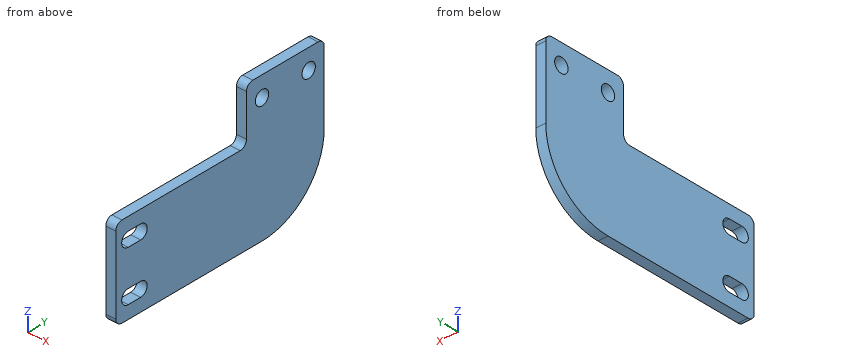
from build123d import *

# Parameters (mm, degrees)
EXTRUDE_1_DEPTH             = 3
EXTRUDE_2_DEPTH             = 3
CUT_EXTRUDE_1_DEPTH         = 3
FILLET_2_R                  = 2
HOLE_WIZARD_4_3_4_3_1_D     = 4.3
HOLE_WIZARD_4_3_4_3_1_DEPTH = 10.1
HOLE_WIZARD_4_3_4_3_1_TIP   = 1.291850331
EXTRUDE_3_DEPTH             = 3
PATTERN_LINEAR_1_COUNT      = 2
PATTERN_LINEAR_1_PITCH      = 24
SKETCH_8_W                  = 24.221203915
SKETCH_8_H                  = 43.975746473
CUT_EXTRUDE_2_DEPTH         = 10
SKETCH_9_W                  = 8.594531195
SKETCH_9_H                  = 29.155429328
CUT_EXTRUDE_3_DEPTH         = 10
FILLET_3_R                  = 2
FILLET_4_R                  = 20


with BuildPart() as part:
    # 草图1 → 凸台-拉伸1 (new body)
    with BuildSketch(Plane(origin=(0, 0, 0), x_dir=(0, 0, -1), z_dir=(1, 0, 0))):
        Polygon((-12.5, 6), (-6, 6), (-6, 61), (6, 61), (6, 6), (12.5, 6), (12.5, -6), (-12.5, -6), align=None)
    extrude(amount=EXTRUDE_1_DEPTH)

    # 草图2 → 凸台-拉伸2 (add)
    with BuildSketch(Plane.ZY):
        Polygon((-6, 61), (-12.5, 6), (12.5, 6), (6, 61), align=None)
    extrude(amount=-EXTRUDE_2_DEPTH)

    # 草图3 → 切除-拉伸1 (cut)
    with BuildSketch(Plane.ZY):
        with BuildLine():
            Line((-5.4, 2), (-5.4, -2))
            ThreePointArc((-5.4, -2), (-7.5, -4.1), (-9.6, -2))
            Line((-9.6, -2), (-9.6, 2))
            ThreePointArc((-9.6, 2), (-7.5, 4.1), (-5.4, 2))
        make_face()
        with BuildLine():
            Line((5.4, 2), (5.4, -2))
            ThreePointArc((5.4, -2), (7.5, -4.1), (9.6, -2))
            Line((9.6, -2), (9.6, 2))
            ThreePointArc((9.6, 2), (7.5, 4.1), (5.4, 2))
        make_face()
    cut_extrude_1 = extrude(amount=-CUT_EXTRUDE_1_DEPTH, mode=Mode.SUBTRACT)

    # 圆角2
    fillet_2_edges = [part.edges().sort_by_distance(p)[0] for p in [
        (1.5, -6, -12.5),
        (1.5, -6, 12.5),
    ]]
    fillet(fillet_2_edges, radius=FILLET_2_R)

    # Ø4.3 (4.3) 直径孔1
    with Locations(Plane.ZY):
        with Locations((0, 56), (0, 41)):
            Hole(HOLE_WIZARD_4_3_4_3_1_D / 2, depth=HOLE_WIZARD_4_3_4_3_1_DEPTH)
            with Locations((0, 0, -(HOLE_WIZARD_4_3_4_3_1_DEPTH + HOLE_WIZARD_4_3_4_3_1_TIP / 2))):  # 118° drill point
                Cone(0, HOLE_WIZARD_4_3_4_3_1_D / 2, HOLE_WIZARD_4_3_4_3_1_TIP, mode=Mode.SUBTRACT)

    # 草图7 → 凸台-拉伸3 (add)
    with BuildSketch(Plane.ZY):
        Polygon((-3.566854944, 61), (-37.5, 61), (-37.5, -6), (-10.5, -6), (-10.5, 36), (-3.566854944, 36), align=None)
    extrude(amount=-EXTRUDE_3_DEPTH)

    # 阵列(线性)1: 切除-拉伸1 ×2
    with Locations(*[(0, 0, -i * PATTERN_LINEAR_1_PITCH) for i in range(1, PATTERN_LINEAR_1_COUNT)]):
        add(cut_extrude_1, mode=Mode.SUBTRACT)

    # 草图8 → 切除-拉伸2 (cut)
    with BuildSketch(Plane.ZY):
        with Locations((1.610601958, 14.012126763)):
            Rectangle(SKETCH_8_W, SKETCH_8_H)
    extrude(amount=-CUT_EXTRUDE_2_DEPTH, mode=Mode.SUBTRACT)

    # 草图9 → 切除-拉伸3 (cut)
    with BuildSketch(Plane.ZY):
        with Locations((10.297265598, 46.422285336)):
            Rectangle(SKETCH_9_W, SKETCH_9_H)
    extrude(amount=-CUT_EXTRUDE_3_DEPTH, mode=Mode.SUBTRACT)

    # 圆角3
    fillet_3_edges = [part.edges().sort_by_distance(p)[0] for p in [
        (1.5, -6, -37.5),
        (1.5, 36, -10.5),
        (1.5, 61, 6),
        (1.5, -6, -10.5),
        (1.5, 36, 6),
    ]]
    fillet(fillet_3_edges, radius=FILLET_3_R)

    # 圆角4
    fillet_4_edges = [part.edges().sort_by_distance(p)[0] for p in [
        (1.5, 61, -37.5),
    ]]
    fillet(fillet_4_edges, radius=FILLET_4_R)


solid = part.part
CAD build for the part. Positions are in the model's coordinates, mm. Give positions to 0.01 mm unless a question says otherwise; leave off trailing zeros. Order: outer loops, then holes, each group sorted by start corner. A loop starts at its lowest first (then second) coordinate and runs counter-clockwise, first axis right, second up. Notation, with made-up numbers: (39.5, 17) - (51.5, 17) arc R19 cw to (51.5, 49) - close; hole circle Ø4 at (75.5, -18.75). An arc over 180 degrees is marked (long way). Answer in a Markdown table with one row per item.
1. Probe probe 1 along Y at (x, z) = (1.6, 0); probe 2 along Z at (x, y) = (1.75, 2); probe 3 along Y at (x, z) = (0.55, -8). List the from-to ranges inside material, lowest first. Write a range as [from, to].
Data:
| item | result |
|---|---|
| probe 1 | y = [36, 38.85], [43.15, 53.85], [58.15, 61] |
| probe 2 | z = [-37.5, -33.6], [-29.4, -18.6], [-14.4, -10.5] |
| probe 3 | y = [36, 61] |
2. Saw through at D-D, the plane z = -16.5. Give the cut face in (x, y), plus the area to 3 significant figures.
Data:
| item | result |
|---|---|
| outline | (0, -6) - (3, -6) - (3, -4.1) - (0, -4.1) - close; (0, 4.1) - (3, 4.1) - (3, 61) - (0, 61) - close |
| area | 176 mm² |
3. Saw through at B-B, the plane z = 0. Give the cut face in (x, y), plus the area to 3 significant figures.
Data:
| item | result |
|---|---|
| outline | (0, 36) - (3, 36) - (3, 38.85) - (0, 38.85) - close; (0, 43.15) - (3, 43.15) - (3, 53.85) - (0, 53.85) - close; (0, 58.15) - (3, 58.15) - (3, 61) - (0, 61) - close |
| area | 49.2 mm² |
4. Saw through at A-A, the plane y = 0. Give the cut face in (x, z), plus the area to 3 significant figures.
Data:
| item | result |
|---|---|
| outline | (0, -37.5) - (3, -37.5) - (3, -33.6) - (0, -33.6) - close; (0, -29.4) - (3, -29.4) - (3, -18.6) - (0, -18.6) - close; (0, -14.4) - (3, -14.4) - (3, -10.5) - (0, -10.5) - close |
| area | 55.8 mm² |
5. Flat gauge pins, fed straight in: pin 1 (1.5 mm diameter, centred on x = 1, y = 1, fed in from +Z); pin 2 (1.5 mm diameter, centred on x = 1, z = -3.5, fed in from -Y). Where does each tip first touch, or does it go through?
Data:
| item | result |
|---|---|
| pin 1 | stops at z = -10.5 |
| pin 2 | stops at y = 36 |
6. Saw through at C-C, the plane x = 0.8. Give the cut face in (y, z).
Data:
| item | result |
|---|---|
| outline | (-6, -35.5) arc R2 ccw to (-4, -37.5) - (41, -37.5) arc R20 ccw to (61, -17.5) - (61, 4) arc R2 ccw to (59, 6) - (38, 6) arc R2 ccw to (36, 4) - (36, -8.5) arc R2 cw to (34, -10.5) - (-4, -10.5) arc R2 ccw to (-6, -12.5) - close; hole (-2, -33.6) - (2, -33.6) arc R2.1 ccw to (2, -29.4) - (-2, -29.4) arc R2.1 ccw to start; hole (-2, -18.6) - (2, -18.6) arc R2.1 ccw to (2, -14.4) - (-2, -14.4) arc R2.1 ccw to start; hole circle Ø4.3 at (41, 0); hole circle Ø4.3 at (56, 0) |
